```python
from build123d import *


with BuildPart() as part:
    # Stepped Bushing Profile → Stepped Bushing Revolve (revolve)
    with BuildSketch(Plane.XY, mode=Mode.PRIVATE) as stepped_bushing_revolve_sk:
        Polygon((-42.407900521, 15), (-42.407900521, 40), (-2.407900521, 40), (-2.407900521, 50), (37.592099479, 50), (37.592099479, 60), (77.592099479, 60), (77.592099479, 70), (117.592099479, 70), (117.592099479, 60), (85.592099479, 60), (85.592099479, 50), (53.592099479, 50), (53.592099479, 40), (21.592099479, 40), (21.592099479, 30), (77.592099479, 30), (77.592099479, 15), align=None)
    revolve(stepped_bushing_revolve_sk.sketch.rotate(Axis((-96.985663619, 0, 0), (1, 0, 0)), 90), axis=Axis((-96.985663619, 0, 0), (1, 0, 0)))


solid = part.part
```
Can you work these out from the model? Positions are in its coordinate system, mm. A direction names the side the tool comes from. Coordinates: 2 decimals unless noted, no trailing zeros. Loops run counter-clockwise (first coordinate to the right, second up) from the corner with the lowest first, then second, coordinate; pieces in that order, holes last. Notation, with made-up numbers: (41, 78) - (96, 78) arc R22 ccw to (96, 105) - close; hole circle Ø11 at (77.5, 61.5). An arc over 180 degrees is marked (long way). Use a Markdown table: item, result.
Item 1: Will these pins go through, and if not, where does the flat tip stop? pin 1 (5 mm diameter, centred on x = 48.5, z = 8.5, fed in from +Y); pin 2 (4 mm diameter, centred on x = 96, z = 29.5, fed in from +Y); pin 3 (12 mm diameter, centred on y = -29.5, z = 45.5, fed in from -X).
Numbers:
| item | result |
|---|---|
| pin 1 | stops at y = 59.7 |
| pin 2 | stops at y = 64.37 |
| pin 3 | stops at x = -2.41 |
Item 2: I want a section at C-C on x = 82.5. Please give me the cut outline in (y, z), and give its area (3 significant figures).
Numbers:
| item | result |
|---|---|
| outline | circle Ø140 at (0, 0); hole circle Ø100 at (0, 0) |
| area | 7,540 mm2 |
Item 3: I want a section at A-A on x = 31.5. Please give me the cut outline in (y, z), and give its area (3 significant figures).
Numbers:
| item | result |
|---|---|
| outline | circle Ø100 at (0, 0); circle Ø60 at (0, 0); hole circle Ø80 at (0, 0); hole circle Ø30 at (0, 0) |
| area | 4,950 mm2 |
Item 4: For faces 1 (the face through (-42.408, -1, -17)), 2 (the face through (69.37, -15.02, 47.69)), 3 (the face through (-2.408, -34, 22)), which set-ups out of +Z, -Z, +X, -X, +Y, -Y let a thin tool reach every point of the face, with its end or its side?
Numbers:
| item | result |
|---|---|
| face 1 | +Z, -Z, -X, +Y, -Y |
| face 2 | +X |
| face 3 | -X |
Item 5: I want a section at D-D on z = -56.5. Please give me the cut outline in (x, y).
Numbers:
| item | result |
|---|---|
| outline | (37.59, -20.19) - (77.59, -20.19) - (77.59, -41.32) - (117.59, -41.32) - (117.59, -20.19) - (85.59, -20.19) - (85.59, 20.19) - (117.59, 20.19) - (117.59, 41.32) - (77.59, 41.32) - (77.59, 20.19) - (37.59, 20.19) - close |
Item 6: We'd pull the mould along Y, two halves only. Please class faces 4 (the face through (117.592, -31, 52)), 5 (the face through (97.872, 68.335, -15.175)), 6 (the face through (49.984, -25.296, 16.128)): released by +Y, released by -Y, zero draft, split by the parting line, or undercut.
Numbers:
| item | result |
|---|---|
| face 4 | zero draft |
| face 5 | split by the parting line |
| face 6 | undercut |
Item 7: I want a section at B-B on z = 33. Please give me the cut outline in (x, y), and give its area (3 significant figures).
Numbers:
| item | result |
|---|---|
| outline | (-42.41, -22.61) - (-2.41, -22.61) - (-2.41, -37.56) - (37.59, -37.56) - (37.59, -50.11) - (77.59, -50.11) - (77.59, -61.73) - (117.59, -61.73) - (117.59, -50.11) - (85.59, -50.11) - (85.59, -37.56) - (53.59, -37.56) - (53.59, -22.61) - (21.59, -22.61) - (21.59, 22.61) - (53.59, 22.61) - (53.59, 37.56) - (85.59, 37.56) - (85.59, 50.11) - (117.59, 50.11) - (117.59, 61.73) - (77.59, 61.73) - (77.59, 50.11) - (37.59, 50.11) - (37.59, 37.56) - (-2.41, 37.56) - (-2.41, 22.61) - (-42.41, 22.61) - close |
| area | 6,700 mm2 |
Item 8: If I drill on probe 1 along Y at (x, z) = (44, 0); probe 2 along Y at (x, z) = (33, 0); probe 3 along Z at (x, y) = (101.5, 1.5), over which ranges is the centre line in solid material (lowest first)? Write a range as from..to.
Numbers:
| item | result |
|---|---|
| probe 1 | y = -60..-40, -30..-15, 15..30, 40..60 |
| probe 2 | y = -50..-40, -30..-15, 15..30, 40..50 |
| probe 3 | z = -69.98..-59.98, 59.98..69.98 |
